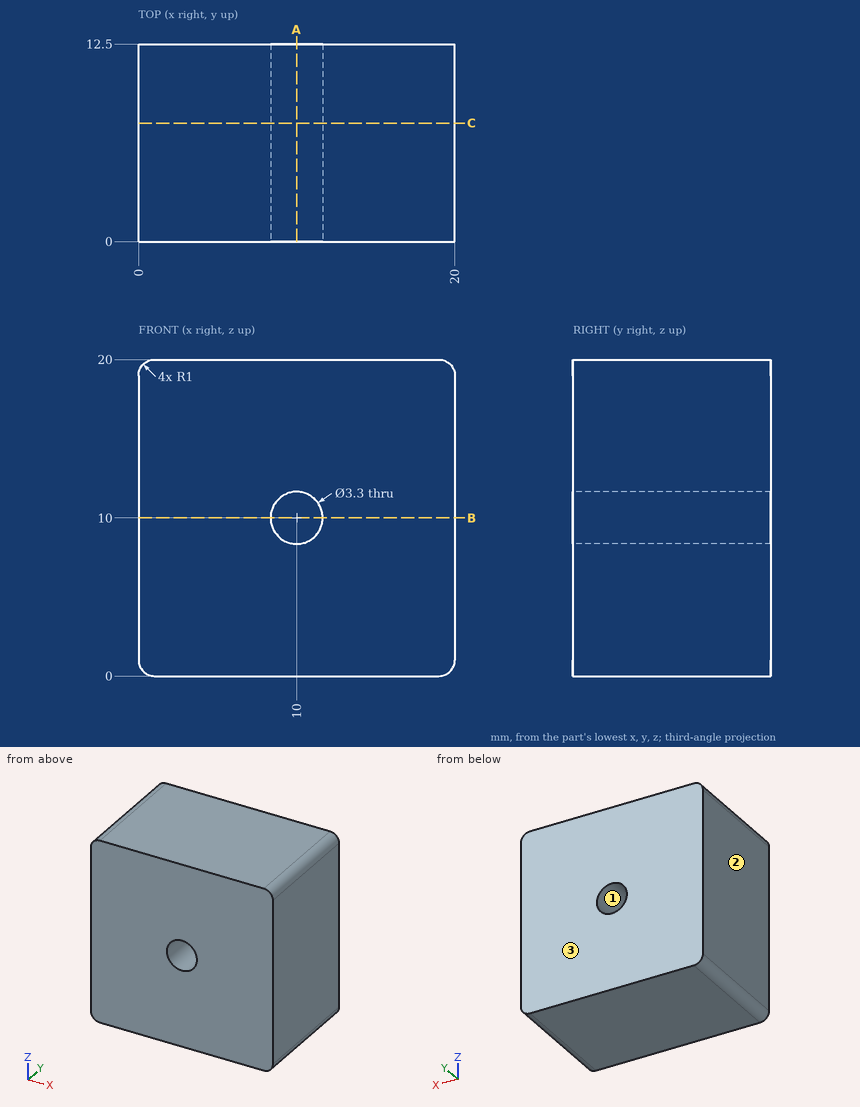
Part print with two shaded views. Sizes in mm from the minimum x, y, z corner. Round coordinates to 2 decimals unless told otherwise and drop trailing zeros. Loops run counter-clockwise (first coordinate to the right, second up) from the corner with the lowest first, then second, coordinate; pieces in that order, holes last.
Item 1: Saw through at A-A (x = 10). List the corners of the cut face in (y, z).
Item 2: Two-plate mould, pull along X, no slides. Class the marked faces 1, 2 and 3: released by +X, released by -X, zero draft, split by the parting line, or undercut.
Item 3: Pin check, flat tip, straight feed: P1, Ø5, axis at y = 9, z = 6.5, coming from the -X side. Stop position of the tip, or through.
Item 4: Drill centre lines: line 1 along Z through (x, y) = (10, 4); line 2 along X through (y, z) = (4.25, 8.75). Where is each one in solid material? Low to high.
Item 5: Saw through at B-B (z = 10). List the corners of the cut face in (x, y).
Item 6: Saw through at C-C (y = 7.5). List the corners of the cut face in (x, z), then the cut area to 3 significant figures.
Worked answers:
1. outline: (0, 0) - (12.5, 0) - (12.5, 8.35) - (0, 8.35) - close; (0, 11.65) - (12.5, 11.65) - (12.5, 20) - (0, 20) - close
2. face 1: undercut
2. face 2: released by -X
2. face 3: zero draft
3. P1: stops at x = 0
4. line 1: z = 0 to 8.35, 11.65 to 20
4. line 2: x = 0 to 8.92, 11.08 to 20
5. outline: (0, 0) - (8.35, 0) - (8.35, 12.5) - (0, 12.5) - close; (11.65, 0) - (20, 0) - (20, 12.5) - (11.65, 12.5) - close
6. outline: (0, 1) arc R1 ccw to (1, 0) - (19, 0) arc R1 ccw to (20, 1) - (20, 19) arc R1 ccw to (19, 20) - (1, 20) arc R1 ccw to (0, 19) - close; hole circle Ø3.3 at (10, 10)
6. area: 391 mm2
